Part model, mm, in its own coordinate system. Face numbers are marked on the shaded views. A direction names the side the tool comes from. Round coordinates to 2 decimals unless told otherwise and drop trailing zeros. Write each loop counter-clockwise with the first axis right and the second up, starting at its lowest first coordinate (ties: lowest second). Pieces come first, ordered by that corner, then holes.
1) Drill centre lines: L1, parallel to Y at x = -17.5, z = 21; L2, parallel to Z at x = 0, y = -21; L3, parallel to Y at x = -8.5, z = 7. Where is each one in solid material? Low to high.
2) Pull direction Z, two halves, no side cores. Call the marked faces 1, 2, 3 and 4: +Z half, -Z half, draft (parallel to the pull), parting line (faces both ways), or undercut.
3) Which spindle directions (+Z, -Z, +X, -X, +Y, -Y) get a long thin tool onto all of the face, cutting with end or side? Do the marked faces 5, 6, 7 and 8. Say none if no direction does.
4) Saw through at A-A on x = -7.5. Write the cut outline in (y, z).
5) Flat gauge pins, fed straight in: pin 1 (4 mm diameter, centred on x = -1, y = 61.5, fed in from -Z); pin 2 (22.5 mm diameter, centred on x = -8.5, z = -49.5, fed in from +Y); pin 3 (23 mm diameter, centred on y = -21.25, z = 36.81, fed in from -X); pin 4 (16 mm diameter, centred on y = -21.25, z = -36.81, fed in from +X). Where does each tip first touch, or does it go through?
6) Saw through at B-B on y = -21.25. Count the separate pieces of the cut face and the enclosed holes in it, and give its area (3 significant figures).
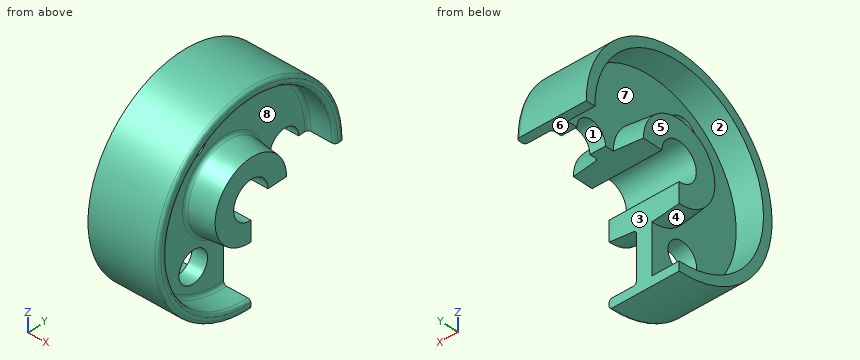
```python
from build123d import *

# Parameters (mm, degrees)
RIM_SLOT_SKETCH_R         = 10
RIM_SLOT_CUT_DEPTH        = 96.949205312
EDGE_FILLET_R2_A_R        = 2
EDGE_FILLET_R2_B_R        = 2
WEB_RELIEF_CUT_DEPTH      = 96.94920538
WEB_RELIEF_CUT_DEPTH_BACK = 96.94920538


with BuildPart() as part:
    # Wheel Profile Sketch → Wheel Body Revolve (revolve)
    with BuildSketch(Plane.XY, mode=Mode.PRIVATE) as wheel_body_revolve_sk:
        Polygon((22.5, 12), (-22.5, 12), (-22.5, 25), (-5, 27), (-5, 59), (-22.5, 59), (-22.5, 65), (22.5, 65), (22.5, 59), (5, 59), (5, 27), (22.5, 25), align=None)
    revolve(wheel_body_revolve_sk.sketch.rotate(Axis((-53.084730572, 0, 0), (1, 0, 0)), 90), axis=Axis((-53.084730572, 0, 0), (1, 0, 0)))

    # Rim Slot Sketch → Rim Slot Cut (cut, through all)
    with BuildSketch(Plane(origin=(5, 0, 0), x_dir=(0, 0, -1), z_dir=(1, 0, 0))):
        with Locations((0, 42.5)):
            Circle(RIM_SLOT_SKETCH_R)
        with Locations((36.806079661, -21.25)):
            Circle(RIM_SLOT_SKETCH_R)
        with Locations((-36.806079661, -21.25)):
            Circle(RIM_SLOT_SKETCH_R)
    extrude(amount=-RIM_SLOT_CUT_DEPTH, mode=Mode.SUBTRACT)

    # Edge Fillet R2 A
    edge_fillet_r2_a_edges = [part.edges().sort_by_distance(p)[0] for p in [
        (22.5, 0, -65),
        (5, 0, -59),
        (5, 0, -27),
    ]]
    fillet(edge_fillet_r2_a_edges, radius=EDGE_FILLET_R2_A_R)

    # Edge Fillet R2 B
    edge_fillet_r2_b_edges = [part.edges().sort_by_distance(p)[0] for p in [
        (22.5, 0, -59),
    ]]
    fillet(edge_fillet_r2_b_edges, radius=EDGE_FILLET_R2_B_R)

    # Web Relief Sketch → Web Relief Cut (cut, two sides: drawn at the far end of the back side and taken through both)
    with BuildSketch(Plane(origin=(5, 0, 0), x_dir=(0, 0, -1), z_dir=(1, 0, 0)).offset(-WEB_RELIEF_CUT_DEPTH_BACK)):
        with BuildLine():
            Line((0, 77.992606611), (0, 0))
            Line((0, 0), (85.280618665, 0))
            ThreePointArc((85.280618665, 0), (62.367801888, 60.567229614), (0, 77.992606611))
        make_face()
    extrude(amount=WEB_RELIEF_CUT_DEPTH + WEB_RELIEF_CUT_DEPTH_BACK, mode=Mode.SUBTRACT)


solid = part.part
```
Completed:
1. L1: y = -61.51 to -55.14, -14.59 to 14.59, 55.14 to 61.51
1. L2: z = -61.51 to -46.8, -26.81 to 26.81, 46.8 to 61.51
1. L3: y = -64.62 to -58.58, -25.66 to -9.75, 9.75 to 25.66, 58.58 to 64.62
2. face 1: -Z half
2. face 2: undercut
2. face 3: draft
2. face 4: undercut
3. face 5: +Z, -Z, -X, +Y, -Y
3. face 6: -Z, +X, -X, +Y
3. face 7: -X
3. face 8: +X
4. outline: (0, -65) - (0, -59) arc R59 cw (long way) to (59, 0) - (65, 0) arc R65 ccw (long way) to start; (0, -26.71) - (0, -12) arc R12 cw (long way) to (12, 0) - (26.71, 0) arc R26.71 ccw (long way) to start
5. pin 1: stops at z = 0
5. pin 2: stops at y = 0
5. pin 3: stops at x = -5
5. pin 4: passes through
6. separate pieces: 3
6. enclosed holes: 0
6. area: 2,320 mm2
